from build123d import *

# Parameters (mm, degrees)
GIB_BODY_EXTRUDE_12MM_DEPTH = 6


with BuildPart() as part:
    # Gib Profile Sketch → Gib Body Extrude 12mm (new, symmetric)
    with BuildSketch(Plane.XY):
        with BuildLine():
            Line((-26, 30.177777778), (0, 30.177777778))
            Line((0, 30.177777778), (0, -63.822222222))
            Line((0, -63.822222222), (-26, -63.822222222))
            ThreePointArc((-26, -63.822222222), (-33.071067812, -60.893290034), (-36, -53.822222222))
            Line((-36, -53.822222222), (-36, -47.822222222))
            Line((-36, -47.822222222), (-22, -47.822222222))
            Line((-22, -47.822222222), (-22, 14.177777778))
            Line((-22, 14.177777778), (-36, 14.177777778))
            Line((-36, 14.177777778), (-36, 20.177777778))
            ThreePointArc((-36, 20.177777778), (-33.071067812, 27.24884559), (-26, 30.177777778))
        make_face()
    extrude(amount=GIB_BODY_EXTRUDE_12MM_DEPTH, both=True)


solid = part.part
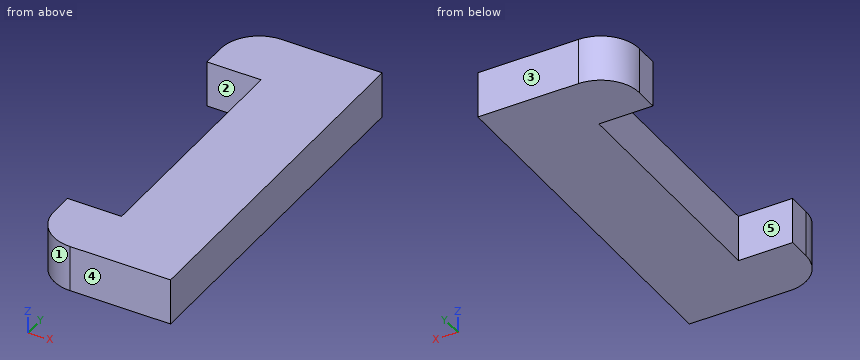
Build history of the part. All positions in model axes, mm. Face numbers are marked on the shaded views. A direction names the side the tool comes from. Round coordinates to 2 decimals unless told otherwise and drop trailing zeros. Loops run counter-clockwise (first coordinate to the right, second up) from the corner with the lowest first, then second, coordinate; pieces in that order, holes last. Notation, with made-up numbers: (19, 59) -> (34, 59) arc R33 cw to (34, 88) -> close; hole circle Ø5 at (16.5, 15). An arc over 180 degrees is marked (long way). Use CSV: the item, a comma, the result in double quotes. Start each with the question number.
Q1. Drill centre lines: L1, parallel to Y at x = -26, z = -5.5; L2, parallel to X at y = 2, z = 0; L3, parallel to Y at x = -29, z = 4.75. Where is each one in solid material? Low to high.
Q2. Flat gauge pin, fed straight in: pin 1 Ø3 at (y, z) = (-29, -1.5) entering from -X. Where does the tip first touch, or does it go through?
Q3. Saw through at B-B on x = -29. Give the cut face in (y, z).
Q4. Which spindle directions (+Z, -Z, +X, -X, +Y, -Y) get a long thin tool onto all of the face, cutting with end or side? Do the marked faces 4 and 5. Say none if no direction does.
Q5. Saw through at C-C on y = -27.5. Give the cut face in (x, z), and give its area (3 significant figures).
Q6. Saw through at A-A on z = 1. Give the cut face in (x, y), and give its area (3 significant figures).
Q7. Mould opens along Y. For the marked faces 1, 2 and 3 say: +Y half, -Y half, draft (parallel to the pull), parting line (faces both ways), or undercut.
Solutions:
1,L1,"y = -63.82 to -47.82, 14.18 to 30.18"
1,L2,"x = -22 to 0"
1,L3,"y = -63.36 to -47.82, 14.18 to 29.72"
2,pin 1,"stops at x = -22"
3,outline,"(-63.36, -6) -> (-47.82, -6) -> (-47.82, 6) -> (-63.36, 6) -> close; (14.18, -6) -> (29.72, -6) -> (29.72, 6) -> (14.18, 6) -> close"
4,face 4,"+Z, -Z, +X, -X, -Y"
4,face 5,"+Z, -Z, -X"
5,outline,"(-22, -6) -> (0, -6) -> (0, 6) -> (-22, 6) -> close"
5,area,"264 mm^2"
6,outline,"(-36, -53.82) arc R10 ccw to (-26, -63.82) -> (0, -63.82) -> (0, 30.18) -> (-26, 30.18) arc R10 ccw to (-36, 20.18) -> (-36, 14.18) -> (-22, 14.18) -> (-22, -47.82) -> (-36, -47.82) -> close"
6,area,"2,470 mm^2"
7,face 1,"-Y half"
7,face 2,"undercut"
7,face 3,"+Y half"
